Input: part model. Units: mm. Frame: model coordinates. A direction names the side the tool comes from. Coordinates: 2 decimals unless noted, no trailing zeros. Write each loop counter-clockwise with the first axis right and the second up, starting at its lowest first coordinate (ties: lowest second). Pieces come first, ordered by that corner, then holes. Notation, with made-up numbers: (8.5, 31) - (64.5, 31) arc R37 cw to (64.5, 68) - close; hole circle Ø8 at (-39, -32). An arc over 180 degrees is marked (long way). Put each result on its own line as item: value. Start each with the question number.
1. Line query: line 1 (Y direction, x = 80, z = -46.9); line 2 (X direction, y = -27, z = -23.5); line 3 (Z direction, x = 92, y = 22). Output: solid intervals per line, ascending.
2. Access query for faces 4 (the flat face through (51, 7, -44)), 5 (the cylindrical face through (55, 0, -47)). Directions: +Z, -Z, +X, -X, +Y, -Y. A direction counts if a zero-diameter tool reaches every point of the face in a straight line with its end or side. Return the directions, or none.
3. Cut plane C-C, the plane x = 50. Return loops of the section in (y, z).
4. Pin query (flat end, axial travel): pin 1 (1.5 mm diameter, centred on x = 33, y = 9.5, fed in from +Z). Return the tip coordinate at first contact, or that it passes through.
5. Cut plane A-A, the plane z = -10. Return loops of the section in (x, y).
6. Pull-direction query (Y, two-part tool) for faces 1 (the flat face through (49, 7, -50)), 2 (the cylindrical face through (75.381, -1.915, -47.042)), 3 (the flat face through (50, -30, -45)); classes: released by +Y, released by -Y, zero draft, split by the parting line, or undercut.
7. Cut plane B-B, the plane z = -30.5. Return loops of the section in (x, y), and give its area (3 significant figures).
8. Cut plane D-D, the plane y = 0. Count the separate pieces of the cut face and the enclosed holes in it, and give its area (3 significant figures).
from build123d import *

# Parameters (mm, degrees)
CHANNEL_BODY_DEPTH      = 30
FLANGE_HOLES_SKETCH_R   = 5
FLANGE_HOLES_DEPTH      = 30
BACK_WALL_HOLES_REACH   = 117.758
BACK_WALL_HOLE_SKETCH_R = 5
CORNER_FILLETS_R5_R     = 5


with BuildPart() as part:
    # Channel Profile Sketch → Channel Body (new, symmetric)
    with BuildSketch(Plane(origin=(0, 0, 0), x_dir=(1, 0, 0), z_dir=(0, 1, 0))):
        Polygon((0, 0), (0, 50), (100, 50), (100, 0), (94, 0), (94, 44), (6, 44), (6, 0), align=None)
    extrude(amount=CHANNEL_BODY_DEPTH, both=True)

    # Flange Holes Sketch → Flange Holes (cut, symmetric)
    with BuildSketch(Plane(origin=(0, 0, -50), x_dir=(-1, 0, 0), z_dir=(0, 0, -1))):
        with Locations((-50, 0)):
            Circle(FLANGE_HOLES_SKETCH_R)
        with Locations((-20, 0)):
            Circle(FLANGE_HOLES_SKETCH_R)
        with Locations((-80, 0)):
            Circle(FLANGE_HOLES_SKETCH_R)
    extrude(amount=FLANGE_HOLES_DEPTH, both=True, mode=Mode.SUBTRACT)

    # Back Wall Holes: up to this face of the body (flat: up to its plane)
    back_wall_holes_end = Plane(part.part.faces().sort_by_distance((0, 0, -25))[0])
    # Back Wall Hole Sketch → Back Wall Holes (cut, up to the picked face)
    with BuildSketch(Plane(origin=(100, 0, 0), x_dir=(0, 0, -1), z_dir=(1, 0, 0)), mode=Mode.PRIVATE) as back_wall_holes_sk1:
        with Locations((10, 0)):
            Circle(BACK_WALL_HOLE_SKETCH_R)
    back_wall_holes_tool1 = split(extrude(back_wall_holes_sk1.sketch, amount=-BACK_WALL_HOLES_REACH, mode=Mode.PRIVATE), bisect_by=back_wall_holes_end, keep=Keep.BOTH, mode=Mode.PRIVATE)
    add(back_wall_holes_tool1.solids().sort_by(Axis((100, 0, -10), (-1, 0, 0)))[0], mode=Mode.SUBTRACT)

    # Corner Fillets R5
    corner_fillets_r5_edges = [part.edges().sort_by_distance(p)[0] for p in [
        (0, 0, -50),
        (100, 0, -50),
    ]]
    fillet(corner_fillets_r5_edges, radius=CORNER_FILLETS_R5_R)


solid = part.part
Report:
1. line 1: y = -30 to -5, 5 to 30
1. line 2: x = 0 to 6, 94 to 100
1. line 3: z = -50 to -44
2. face 4: +Z, +Y, -Y
2. face 5: +Z, -Z
3. outline: (-30, -50) - (-5, -50) - (-5, -44) - (-30, -44) - close; (5, -50) - (30, -50) - (30, -44) - (5, -44) - close
4. pin 1: stops at z = -44
5. outline: (0, -30) - (6, -30) - (6, -5) - (0, -5) - close; (0, 5) - (6, 5) - (6, 30) - (0, 30) - close; (94, -30) - (100, -30) - (100, -5) - (94, -5) - close; (94, 5) - (100, 5) - (100, 30) - (94, 30) - close
6. face 1: zero draft
6. face 2: undercut
6. face 3: released by -Y
7. outline: (0, -30) - (6, -30) - (6, 30) - (0, 30) - close; (94, -30) - (100, -30) - (100, 30) - (94, 30) - close
7. area: 720 mm^2
8. separate pieces: 6
8. enclosed holes: 0
8. area: 817 mm^2
